Source: CAD feature listing. Evaluate the final solid. Frame: model axes, mm. Face numbers are marked on the shaded views. Coordinates: 2 decimals unless noted, no trailing zeros. Write each loop counter-clockwise with the first axis right and the second up, starting at its lowest first coordinate (ties: lowest second). Pieces come first, ordered by that corner, then holes. Notation, with made-up numbers: (-7.75, 39) - (-3.75, 39) arc R27 ccw to (-3.75, 64) - close; hole circle Ø8 at (53.5, 23.25). An arc over 180 degrees is marked (long way). One line per item, written item: value.
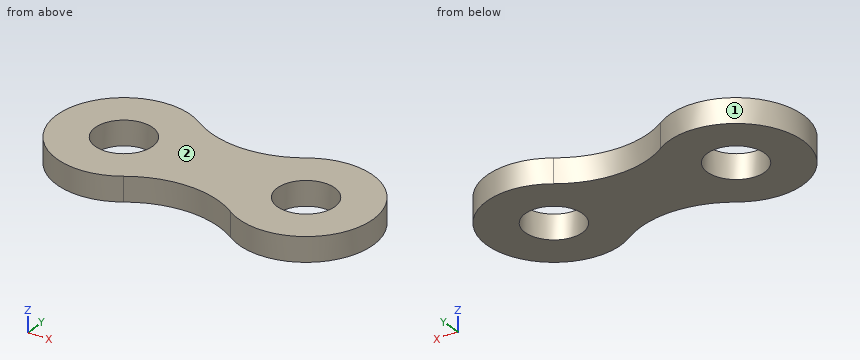
from build123d import *

# Parameters (mm, degrees)
SKETCH1_R           = 3
BOSS_EXTRUDE1_DEPTH = 2.55


with BuildPart() as part:
    # Sketch1 → Boss-Extrude1 (new body)
    with BuildSketch(Plane.XY):
        with BuildLine():
            ThreePointArc((3.922058824, 5.798056104), (-7, 0), (3.922058824, -5.798056104))
            ThreePointArc((3.922058824, -5.798056104), (9.525, -4.080993395), (15.127941176, -5.798056104))
            ThreePointArc((15.127941176, -5.798056104), (26.05, 0), (15.127941176, 5.798056104))
            ThreePointArc((15.127941176, 5.798056104), (9.525, 4.080993395), (3.922058824, 5.798056104))
        make_face()
        Circle(SKETCH1_R, mode=Mode.SUBTRACT)
        with Locations((19.05, 0)):
            Circle(SKETCH1_R, mode=Mode.SUBTRACT)
    extrude(amount=BOSS_EXTRUDE1_DEPTH)


solid = part.part
1) Section query B-B on x = 0. Output: boundary loops of the cut face in (y, z), then the cut area to 3 significant figures.
Values found:
outline: (-7, 0) - (-3, 0) - (-3, 2.55) - (-7, 2.55) - close; (3, 0) - (7, 0) - (7, 2.55) - (3, 2.55) - close
area: 20.4 mm2
2) Draft query along X for the marked faces 1 and 2. Return one class per face: released by +X, released by -X, zero draft, split by the parting line, or undercut.
Values found:
face 1: undercut
face 2: zero draft
3) Material intervals for line 1 (X direction, y = 2.25, z = 0.45); line 2 (Y direction, x = 0, z = 1.7); line 3 (X direction, y = 2.75, z = 1.5), sorted ascending.
Values found:
line 1: -6.63 to -1.98, 1.98 to 17.07, 21.03 to 25.68
line 2: -7 to -3, 3 to 7
line 3: -6.44 to -1.2, 1.2 to 17.85, 20.25 to 25.49
4) Section query D-D on x = 17. Output: boundary loops of the cut face in (y, z).
Values found:
outline: (-6.69, 0) - (-2.19, 0) - (-2.19, 2.55) - (-6.69, 2.55) - close; (2.19, 0) - (6.69, 0) - (6.69, 2.55) - (2.19, 2.55) - close
5) Section query C-C on z = 0.3. Output: boundary loops of the cut face in (x, y) (3 decimals), then the cut area to 3 significant figures.
Values found:
outline: (3.922, -5.798) arc R10 cw to (15.128, -5.798) arc R7 ccw (long way) to (15.128, 5.798) arc R10 cw to (3.922, 5.798) arc R7 ccw (long way) to start; hole circle Ø6 at (0, 0); hole circle Ø6 at (19.05, 0)
area: 305 mm2
6) Contact query for a flat-ended pin moving along its axis: P1, Ø5, axis at x = 0, y = 0, coming from the +Z side. Output: stop coordinate, or through.
Values found:
P1: through
7) Section query A-A on y = 0. Output: boundary loops of the cut face in (x, z), then the cut area to 3 significant figures.
Values found:
outline: (-7, 0) - (-3, 0) - (-3, 2.55) - (-7, 2.55) - close; (3, 0) - (16.05, 0) - (16.05, 2.55) - (3, 2.55) - close; (22.05, 0) - (26.05, 0) - (26.05, 2.55) - (22.05, 2.55) - close
area: 53.7 mm2
